```python
from build123d import *

# Parameters (mm, degrees)
FRONT_FLANGE_SKETCH_W      = 50
FRONT_FLANGE_SKETCH_H      = 50
FRONT_FLANGE_50X50X5_DEPTH = 5
BODY_BLOCK_SKETCH_W        = 40
BODY_BLOCK_SKETCH_H        = 40
BODY_BLOCK_40X40X55_DEPTH  = 55
REAR_FLANGE_SKETCH_W       = 50
REAR_FLANGE_SKETCH_H       = 50
REAR_FLANGE_5MM_DEPTH      = 5
OBROUND_TONGUE_DEPTH       = 25
TONGUE_SLOT_CUT_DEPTH      = 108.819293264
TONGUE_ROOT_FILLET_R2_R    = 2
TONGUE_EDGE_FILLET_R0_5_R  = 0.5
TONGUE_HOLE_SKETCH_R       = 4.75949031
TONGUE_CROSS_HOLE_DEPTH    = 100.829855254


with BuildPart() as part:
    # Front Flange Sketch → Front Flange 50x50x5 (new body)
    with BuildSketch(Plane.XY):
        with Locations((25, 25)):
            Rectangle(FRONT_FLANGE_SKETCH_W, FRONT_FLANGE_SKETCH_H)
    extrude(amount=FRONT_FLANGE_50X50X5_DEPTH)

    # Body Block Sketch → Body Block 40x40x55 (add)
    with BuildSketch(Plane.XY.offset(5)):
        with Locations((25, 25)):
            Rectangle(BODY_BLOCK_SKETCH_W, BODY_BLOCK_SKETCH_H)
    extrude(amount=BODY_BLOCK_40X40X55_DEPTH)

    # Rear Flange Sketch → Rear Flange 5mm (add)
    with BuildSketch(Plane.XY.offset(60)):
        with Locations((25, 25)):
            Rectangle(REAR_FLANGE_SKETCH_W, REAR_FLANGE_SKETCH_H)
    extrude(amount=REAR_FLANGE_5MM_DEPTH)

    # Tongue Profile Sketch → Obround Tongue (add)
    with BuildSketch(Plane(origin=(45, 0, 0), x_dir=(0, 0, -1), z_dir=(1, 0, 0))):
        with BuildLine():
            Line((-47.5, 29), (-17.5, 29))
            ThreePointArc((-17.5, 29), (-13.5, 25), (-17.5, 21))
            Line((-17.5, 21), (-47.5, 21))
            ThreePointArc((-47.5, 21), (-51.5, 25), (-47.5, 29))
        make_face()
    extrude(amount=OBROUND_TONGUE_DEPTH)

    # Tongue Slot Sketch → Tongue Slot Cut (cut, through all)
    with BuildSketch(Plane(origin=(70, 0, 0), x_dir=(0, 0, -1), z_dir=(1, 0, 0))):
        with BuildLine():
            Line((-47.5, 22.5), (-17.5, 22.5))
            ThreePointArc((-17.5, 22.5), (-15, 25), (-17.5, 27.5))
            Line((-17.5, 27.5), (-47.5, 27.5))
            ThreePointArc((-47.5, 27.5), (-50, 25), (-47.5, 22.5))
        make_face()
    extrude(amount=-TONGUE_SLOT_CUT_DEPTH, mode=Mode.SUBTRACT)

    # Tongue Root Fillet R2
    tongue_root_fillet_r2_edges = [part.edges().sort_by_distance(p)[0] for p in [
        (45, 29, 32.5),
        (45, 25, 13.5),
        (45, 21, 32.5),
        (45, 25, 51.5),
    ]]
    fillet(tongue_root_fillet_r2_edges, radius=TONGUE_ROOT_FILLET_R2_R)

    # Tongue Edge Fillet R0.5
    tongue_edge_fillet_r0_5_edges = [part.edges().sort_by_distance(p)[0] for p in [
        (70, 21, 32.5),
        (70, 25, 13.5),
        (70, 25, 51.5),
        (70, 29, 32.5),
    ]]
    fillet(tongue_edge_fillet_r0_5_edges, radius=TONGUE_EDGE_FILLET_R0_5_R)

    # Tongue Hole Sketch → Tongue Cross Hole (cut, through all)
    with BuildSketch(Plane.XZ.offset(-21)):
        with Locations((58.25, 32.5)):
            Circle(TONGUE_HOLE_SKETCH_R)
    extrude(amount=-TONGUE_CROSS_HOLE_DEPTH, mode=Mode.SUBTRACT)


solid = part.part
```
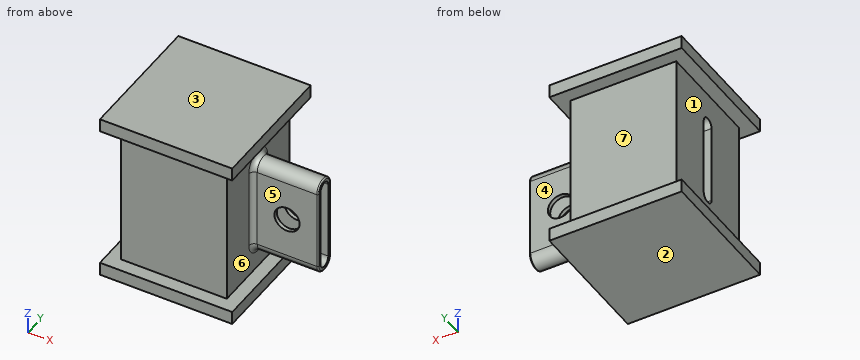
Geometry check sheet. Reference: the model listing, model coordinates, mm. Face numbers are marked on the shaded views. A direction names the side the tool comes from. Coordinates: 2 decimals unless noted, no trailing zeros. Loops run counter-clockwise (first coordinate to the right, second up) from the corner with the lowest first, then second, coordinate; pieces in that order, holes last. Notation, with made-up numbers: (83.5, 3.25) -> (110.5, 3.25) arc R17 ccw to (110.5, 35.25) -> close; hole circle Ø1 at (67, -8.5). An arc over 180 degrees is marked (long way). Put each result on its own line as item: value.
1) Cross-section at C-C on y = 25. Record the boundary of the cut face in (x, z), plus the area to 3 significant figures.
Result set:
outline: (0, 0) -> (50, 0) -> (50, 5) -> (45, 5) -> (45, 11.5) arc R2 cw to (47, 13.5) -> (69.5, 13.5) arc R0.5 ccw to (70, 14) -> (70, 15) -> (5, 15) -> (5, 5) -> (0, 5) -> close; (0, 60) -> (5, 60) -> (5, 50) -> (70, 50) -> (70, 51) arc R0.5 ccw to (69.5, 51.5) -> (47, 51.5) arc R2 cw to (45, 53.5) -> (45, 60) -> (50, 60) -> (50, 65) -> (0, 65) -> close
area: 1,380 mm^2
2) Thickness scan on line 1 (Y direction, x = 63, z = 36.5); line 2 (Z direction, x = 49, y = 9); line 3 (Y direction, x = 39.5, z = 26.5). Record the ranges inside material, lowest first.
Result set:
line 1: y = 21 to 22.5, 27.5 to 29
line 2: z = 0 to 5, 60 to 65
line 3: y = 5 to 22.5, 27.5 to 45
3) Cross-section at B-B on z = 30.5. Record the boundary of the cut face in (x, y).
Result set:
outline: (5, 5) -> (45, 5) -> (45, 19) arc R2 cw to (47, 21) -> (53.93, 21) -> (53.93, 22.5) -> (5, 22.5) -> close; (5, 27.5) -> (53.93, 27.5) -> (53.93, 29) -> (47, 29) arc R2 cw to (45, 31) -> (45, 45) -> (5, 45) -> close; (62.57, 21) -> (69.5, 21) arc R0.5 ccw to (70, 21.5) -> (70, 22.5) -> (62.57, 22.5) -> close; (62.57, 27.5) -> (70, 27.5) -> (70, 28.5) arc R0.5 ccw to (69.5, 29) -> (62.57, 29) -> close
4) Cross-section at D-D on x = 37.5. Record the boundary of the cut face in (y, z), plus the area to 3 significant figures.
Result set:
outline: (0, 0) -> (50, 0) -> (50, 5) -> (45, 5) -> (45, 60) -> (50, 60) -> (50, 65) -> (0, 65) -> (0, 60) -> (5, 60) -> (5, 5) -> (0, 5) -> close; hole (22.5, 17.5) arc R2.5 ccw to (27.5, 17.5) -> (27.5, 47.5) arc R2.5 ccw to (22.5, 47.5) -> close
area: 2,530 mm^2
5) Release check for a two-part mould opening along Z. For the marked faces 1, 2 and 3 record: released by +Z, released by -Z, zero draft, split by the parting line, or undercut.
Result set:
face 1: undercut
face 2: released by -Z
face 3: released by +Z
6) Cross-section at A-A on x = 58.25. Record the boundary of the cut face in (y, z).
Result set:
outline: (21, 17.5) arc R4 ccw to (29, 17.5) -> (29, 27.74) -> (27.5, 27.74) -> (27.5, 17.5) arc R2.5 cw to (22.5, 17.5) -> (22.5, 27.74) -> (21, 27.74) -> close; (21, 37.26) -> (22.5, 37.26) -> (22.5, 47.5) arc R2.5 cw to (27.5, 47.5) -> (27.5, 37.26) -> (29, 37.26) -> (29, 47.5) arc R4 ccw to (21, 47.5) -> close
7) Gauge pin test, flat ends, axial feed: pin 1 Ø5.5 at (y, z) = (21.5, 3) entering from +X; pin 2 Ø8.5 at (x, z) = (58.25, 32.5) entering from +Y; pin 3 Ø5 at (y, z) = (9, 10.5) entering from -X; pin 4 Ø1 at (y, z) = (39.5, 7.5) entering from +X. Record the tip position at first contact, or that the pin passes through.
Result set:
pin 1: stops at x = 50
pin 2: passes through
pin 3: stops at x = 5
pin 4: stops at x = 45
8) Tool access check on the marked faces 4, 5, 6 and 7. Record the directions out of +Z, -Z, +X, -X, +Y, -Y that give a thin tool (end or side, any length) a straight path to the whole face; none if there is none.
Result set:
face 4: +X, +Y
face 5: +X, -Y
face 6: +X
face 7: +X, -X, +Y
